Work out the finished part from the listing and answer in its coordinate system (mm). Face numbers are marked on the shaded views. A direction names the side the tool comes from. Coordinates: 2 decimals unless noted, no trailing zeros. Order: outer loops, then holes, each group sorted by start corner. A loop starts at its lowest first (then second) coordinate and runs counter-clockwise, first axis right, second up. Notation, with made-up numbers: M 72,66.5 L 118,66.5 A36 cw 118,100.5 Z; hole C 49.25,-12 d7. An arc over 180 degrees is marked long. Answer in a Markdown table with one row per item. Add a question column.
Item 1: The part is cut by section B-B (z = 32). Write down the section's boundary in (x, y), then the cut area to 3 significant figures.
Item 2: The part is cut by section D-D (x = -47). Write down the section's boundary in (y, z).
Item 3: The part is cut by section C-C (x = 35.5). Write down the section's boundary in (y, z).
Item 4: The mould has two halves that part along X. Classify the marked faces 5, 6, 7 and 8: released by +X, released by -X, zero draft, split by the parting line, or undercut.
Item 5: Which of the six approach directions +Z, -Z, +X, -X, +Y, -Y give full straight-line access (tool end or side, diameter ignored) to the marked faces 1, 2, 3 and 4?
Item 6: Consider line 1 (Y direction, x = 54, z = 10); line 2 (Y direction, x = -19, z = 24.5); line 3 (Y direction, x = 20, z = 33). Determine where each line is inside the solid, lowest interval first. Write a range as from..to.
Item 7: The part is cut by section A-A (y = 0). Write down the section's boundary in (x, z), then the cut area to 3 significant figures.
Item 8: Flat-ended cylindrical pins translate along their axes: pin 1 Ø1.5 at (y, z) = (18.5, 31) entering from +X; pin 2 Ø12 at (x, z) = (-44.5, 28) entering from +Y; pin 3 Ø19.5 at (x, y) = (53, 49.5) entering from +Z. Find the tip coordinate at first contact, or state that the pin passes through.
from build123d import *

# Parameters (mm, degrees)
LINK_PLATE_DEPTH          = 52
LINK_SLOT_DEPTH           = 52
PIVOT_BOSS_DEPTH          = 34
PIVOT_PIN_HOLE_SKETCH_R   = 4
PIVOT_PIN_HOLE_DEPTH      = 34
SUPPORT_RIB_10MM_REACH    = 145.698
SUPPORT_RIB_SKETCH_WALL_W = 421.148756116
SUPPORT_RIB_SKETCH_WALL_H = 10
EDGE_FILLETS_R15_R        = 15


with BuildPart() as part:
    # Link Plate Outline Sketch → Link Plate (new body)
    with BuildSketch(Plane.XY):
        with BuildLine():
            Line((-54, 34), (54, 34))
            ThreePointArc((54, 34), (88, 0), (54, -34))
            Line((54, -34), (-54, -34))
            ThreePointArc((-54, -34), (-88, 0), (-54, 34))
        make_face()
    extrude(amount=LINK_PLATE_DEPTH)

    # Link Slot Sketch → Link Slot (cut)
    with BuildSketch(Plane.XY.offset(52)):
        with BuildLine():
            Line((-54, 15), (54, 15))
            ThreePointArc((54, 15), (69, 0), (54, -15))
            Line((54, -15), (-54, -15))
            ThreePointArc((-54, -15), (-69, 0), (-54, 15))
        make_face()
    extrude(amount=-LINK_SLOT_DEPTH, mode=Mode.SUBTRACT)

    # Pivot Boss Sketch → Pivot Boss (add)
    with BuildSketch(Plane.XY):
        with BuildLine():
            Line((29, 76), (29, 34))
            Line((29, 34), (29, 18.031591918))
            Line((29, 18.031591918), (79, 18.031591918))
            Line((79, 18.031591918), (79, 76))
            ThreePointArc((79, 76), (54, 101), (29, 76))
        make_face()
    extrude(amount=PIVOT_BOSS_DEPTH)

    # Pivot Pin Hole Sketch → Pivot Pin Hole (cut)
    with BuildSketch(Plane.XY.offset(34)):
        with Locations((54, 76)):
            Circle(PIVOT_PIN_HOLE_SKETCH_R)
    extrude(amount=-PIVOT_PIN_HOLE_DEPTH, mode=Mode.SUBTRACT)

    # Support Rib Sketch wall → Support Rib 10mm (add, up to next)
    with BuildSketch(Plane(origin=(-15.293433294, 63.226194681, 0), x_dir=(0.855125243419, 0.518421467599, 0), z_dir=(-0.518421467599, 0.855125243419, 0)), mode=Mode.PRIVATE) as support_rib_10mm_sk1:
        with Locations((0, -5)):
            Rectangle(SUPPORT_RIB_SKETCH_WALL_W, SUPPORT_RIB_SKETCH_WALL_H)
    support_rib_10mm_tool1 = extrude(support_rib_10mm_sk1.sketch, amount=-SUPPORT_RIB_10MM_REACH, mode=Mode.PRIVATE) - part.part
    add(support_rib_10mm_tool1.solids().sort_by_distance((-15.293433294, 63.226194681, 0))[0])

    # Edge Fillets R15
    edge_fillets_r15_edges = [part.edges().sort_by_distance(p)[0] for p in [
        (29, 34, 22),
    ]]
    fillet(edge_fillets_r15_edges, radius=EDGE_FILLETS_R15_R)


solid = part.part
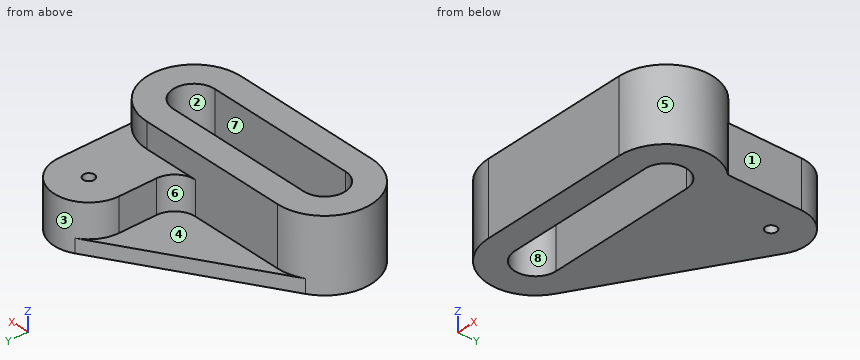
Reply:
| question | item | result |
|---|---|---|
| 1 | outline | M -54,-34 L 54,-34 A34 ccw 79,23.04 L 79,76 A25 ccw 29,76 L 29,49 A15 cw 14,34 L -54,34 A34 ccw Z; hole M -54,-15 L 54,-15 A15 ccw 54,15 L -54,15 A15 ccw Z; hole C 54,76 d8 |
| 1 | area | 10,200 mm2 |
| 2 | outline | M -34,0 L -15,0 L -15,52 L -34,52 Z; M 15,0 L 44,0 L 44,10 L 34,10 L 34,52 L 15,52 Z |
| 3 | outline | M -34,0 L -15,0 L -15,52 L -34,52 Z; M 15,0 L 94.02,0 L 94.02,10 L 92.82,10 L 92.82,34 L 34,34 L 34,52 L 15,52 Z |
| 4 | face 5 | released by +X |
| 4 | face 6 | released by -X |
| 4 | face 7 | undercut |
| 4 | face 8 | undercut |
| 5 | face 1 | +Z, -Z, +X, +Y |
| 5 | face 2 | +Z, -Z |
| 5 | face 3 | +Z, +Y |
| 5 | face 4 | +Z, -X, +Y |
| 6 | line 1 | y = -34..-15, 15..72, 80..101 |
| 6 | line 2 | y = -34..-15, 15..34 |
| 6 | line 3 | y = -34..-15, 15..35.25 |
| 7 | outline | M -88,0 L -69,0 L -69,52 L -88,52 Z; M 69,0 L 88,0 L 88,52 L 69,52 Z |
| 7 | area | 1,980 mm2 |
| 8 | pin 1 | stops at x = 83 |
| 8 | pin 2 | stops at y = 34 |
| 8 | pin 3 | stops at z = 34 |
